Check sheet for the drawn part. Datum: minimum x, y, z corner. Units: mm. A direction names the side the tool comes from. Coordinates: 2 decimals unless noted, no trailing zeros. Loops run counter-clockwise (first coordinate to the right, second up) from the corner with the lowest first, then second, coordinate; pieces in that order, holes last. Notation, with made-up numbers: (-14.75, -35) - (38.25, -35) arc R11 ccw to (38.25, -19) - close; hole circle Ø8 at (-6, 0). An arc over 180 degrees is marked (long way). Answer as a JSON object with one key per item and string values. Group by question number.
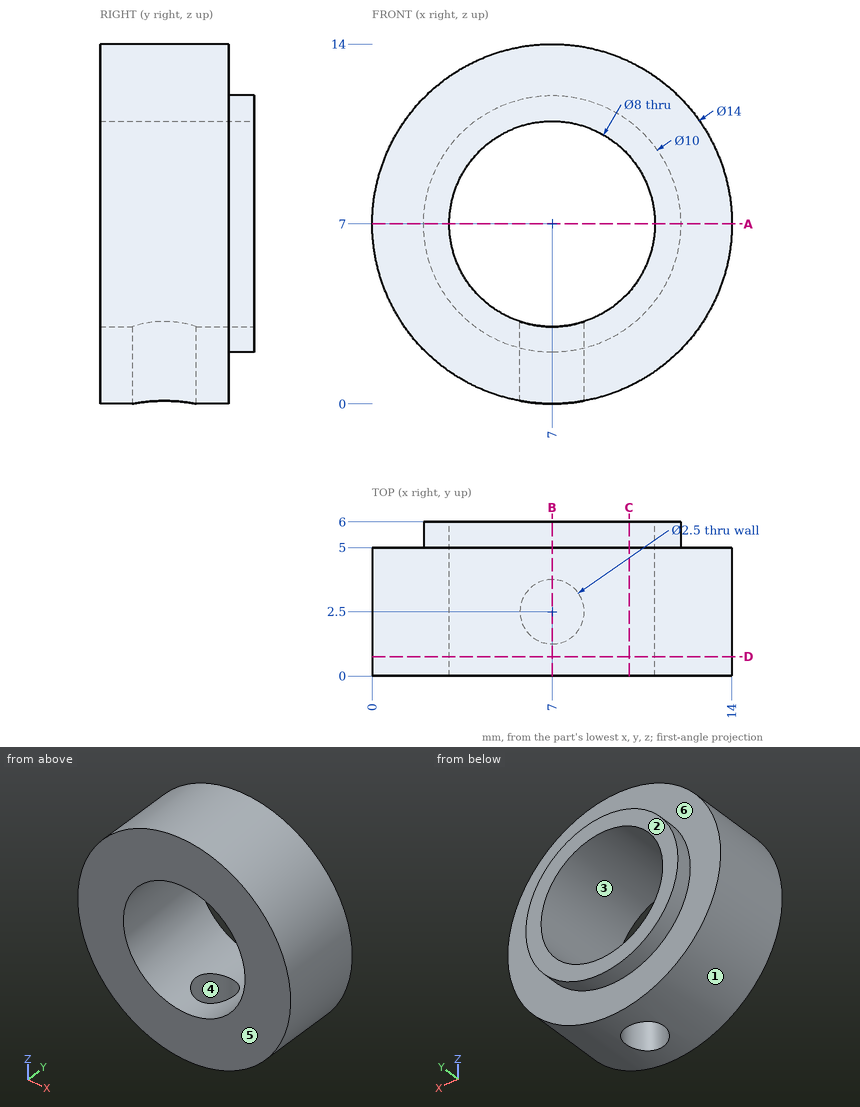
1. Material ranges on line 1 (X direction, y = 2.5, z = 7); line 2 (Y direction, x = 8.75, z = 2.25); line 3 (X direction, y = 1.75, z = 2.75), recorded low to high.
2. Gauge pin test, flat ends, axial feed: pin 1 (1 mm diameter, centred on x = 9, y = 3, fed in from -Z); pin 2 (6 mm diameter, centred on x = 1.5, z = 5.5, fed in from +Y); pin 3 (1 mm diameter, centred on y = 3, z = 6, fed in from -X); pin 4 (2 mm diameter, centred on y = 3.5, z = 2.5, fed in from -X). Record the tip position at first contact, or that the pin passes through.
3. Access from +Z, -Z, +X, -X, +Y, -Y to the whole of each face (thin tool, end or side, straight path). Record for the marked faces 4, 5 and 6.
4. Sectioned sample at B-B on x = 7. Record the cut outline in (y, z).
5. Sectioned sample at C-C on x = 10. Record the cut outline in (y, z), plus the area to 3 significant figures.
6. Release check for a two-part mould opening along Z. For the marked faces 1, 2 and 3 record: released by +Z, released by -Z, zero draft, split by the parting line, or undercut.
7. Sectioned sample at A-A on z = 7. Record the cut outline in (x, y), plus the area to 3 significant figures.
8. Sectioned sample at D-D on y = 0.75. Record the cut outline in (x, z), plus the area to 3 significant figures.
Answers follow:
{
 "1": {"line 1": "x = 0 to 3, 11 to 14", "line 2": "y = 0 to 5", "line 3": "x = 1.44 to 6, 8 to 12.56"},
 "2": {"pin 1": "stops at z = 0.16", "pin 2": "stops at y = 6", "pin 3": "stops at x = 0.02", "pin 4": "stops at x = 0.94"},
 "3": {"face 4": "-Z", "face 5": "+Z, -Z, +X, -X, -Y", "face 6": "+Y"},
 "4": {"outline": "(0, 0) - (1.25, 0) - (1.25, 3) - (0, 3) - close; (0, 11) - (6, 11) - (6, 12) - (5, 12) - (5, 14) - (0, 14) - close; (3.75, 0) - (5, 0) - (5, 2) - (6, 2) - (6, 3) - (3.75, 3) - close"},
 "5": {"outline": "(0, 0.68) - (5, 0.68) - (5, 3) - (6, 3) - (6, 4.35) - (0, 4.35) - close; (0, 9.65) - (6, 9.65) - (6, 11) - (5, 11) - (5, 13.32) - (0, 13.32) - close", "area": "39.5 mm^2"},
 "6": {"face 1": "split by the parting line", "face 2": "zero draft", "face 3": "undercut"},
 "7": {"outline": "(0, 0) - (3, 0) - (3, 6) - (2, 6) - (2, 5) - (0, 5) - close; (11, 0) - (14, 0) - (14, 5) - (12, 5) - (12, 6) - (11, 6) - close", "area": "32.0 mm^2"},
 "8": {"outline": "circle Ø14 at (7, 7); hole circle Ø8 at (7, 7)", "area": "104 mm^2"}
}
